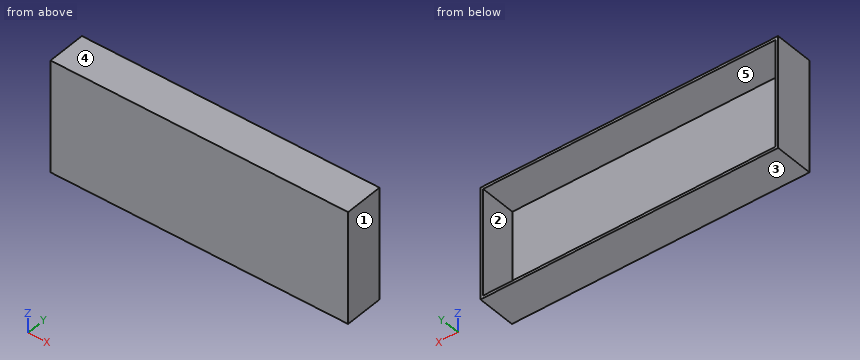
from build123d import *

# Parameters (mm, degrees)
SKETCH1_W           = 690
SKETCH1_H           = 260
BOSS_EXTRUDE1_DEPTH = 90
SHELL1_T            = -6


with BuildPart() as part:
    # Sketch1 → Boss-Extrude1 (new body)
    with BuildSketch(Plane(origin=(0, 0, 0), x_dir=(1, 0, 0), z_dir=(0, 1, 0))):
        Rectangle(SKETCH1_W, SKETCH1_H)
    extrude(amount=BOSS_EXTRUDE1_DEPTH)

    # Shell1
    shell1_openings = [part.faces().sort_by_distance(p)[0] for p in [
        (0, 90, 0),
    ]]
    offset(amount=SHELL1_T, openings=shell1_openings, kind=Kind.INTERSECTION)


solid = part.part
Read the model definition and answer for the solid it produces. Units are mm, in the model's axes. Face numbers are marked on the shaded views. A direction names the side the tool comes from. Coordinates: 2 decimals unless noted, no trailing zeros. Loops run counter-clockwise (first coordinate to the right, second up) from the corner with the lowest first, then second, coordinate; pieces in that order, holes last.
Q1. Which of the six approach directions +Z, -Z, +X, -X, +Y, -Y give full straight-line access (tool end or side, diameter ignored) to the marked faces 4 and 5?
Q2. The part is cut by section A-A on y = 51. Write down the section's boundary in (x, z), and give its area (3 significant figures).
Q3. The mould has two halves that part along Z. Classify the marked faces 1, 2 and 3: +Z half, -Z half, draft (parallel to the pull), parting line (faces both ways), or undercut.
Q4. The part is cut by section C-C on z = -43. Write down the section's boundary in (x, y).
Q5. The part is cut by section B-B on x = -6. Write down the section's boundary in (y, z).
Q6. Consider probe 1 along X at (y, z) = (53.5, 61); probe 2 along Z at (x, y) = (-219, 62); probe 3 along Y at (x, z) = (137.5, -26). Determine where each line is inside the solid, lowest interval first.
Q7. Each of these flat-tipped pins is pushed along its axis until it touches: pin 1 Ø10 at (x, z) = (37, -29) entering from +Y; pin 2 Ø1 at (x, z) = (41.5, -32.5) entering from -Y. Where does it stop, or does it pass through?
Results below:
1. face 4: +Z, +X, -X, +Y, -Y
1. face 5: +Y
2. outline: (-345, -130) - (345, -130) - (345, 130) - (-345, 130) - close; hole (-339, -124) - (339, -124) - (339, 124) - (-339, 124) - close
2. area: 11,300 mm2
3. face 1: draft
3. face 2: undercut
3. face 3: -Z half
4. outline: (-345, 0) - (345, 0) - (345, 90) - (339, 90) - (339, 6) - (-339, 6) - (-339, 90) - (-345, 90) - close
5. outline: (0, -130) - (90, -130) - (90, -124) - (6, -124) - (6, 124) - (90, 124) - (90, 130) - (0, 130) - close
6. probe 1: x = -345 to -339, 339 to 345
6. probe 2: z = -130 to -124, 124 to 130
6. probe 3: y = 0 to 6
7. pin 1: stops at y = 6
7. pin 2: stops at y = 0
